Answer from the drawing. Dimensions are ordinates in mm from the lowest x, y and z of the part. A direction names the side the tool comes from. Round coordinates to 2 decimals unless told otherwise and drop trailing zeros. Loops run counter-clockwise (first coordinate to the right, second up) from the corner with the lowest first, then second, coordinate; pieces in that order, holes last.
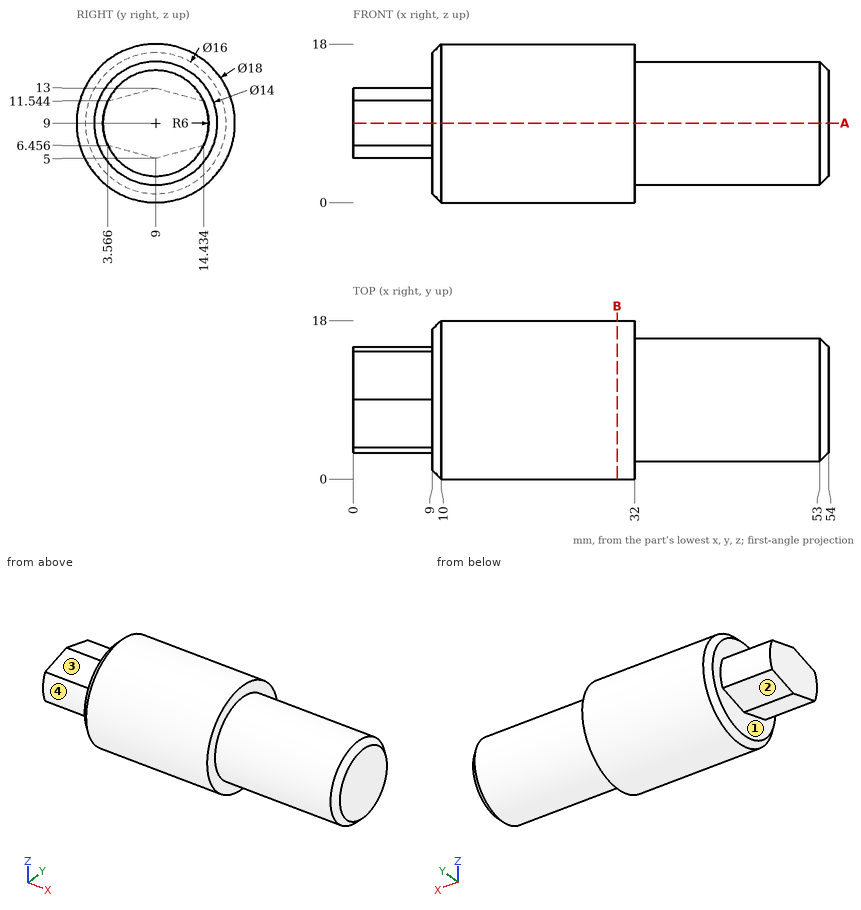
Item 1: Section A-A, the plane z = 9 is taken. Give the vertices of the cut face in (x, y).
Item 2: Straight lines are drawn through the part: line 1 (X direction, y = 3.75, z = 3); line 2 (X direction, y = 9, z = 13.25); line 3 (Y direction, x = 23.5, z = 3). For each, find the intervals that lie inside material, in ascending order.
Item 3: Section B-B, the plane x = 30 is taken. Give the vertices of the cut face in (y, z).
Item 4: For the marked faces 1, 2, 3 and 4, determine the directions among +Z, -Z, +X, -X, +Y, -Y from which every point of the face is accessible in a straight line to the end or side of a thin tool.
Item 5: Each of these flat-tipped pins is pushed along its axis until it touches: P1, Ø3, axis at y = 11, z = 12, coming from the -X side; P2, Ø5, axis at x = 19, y = 3, coming from the +Z side; P3, Ø4, axis at x = 8.5, y = 3, coming from the +Z side; P4, Ø5, axis at x = 30, z = 6, coming from the -Y side. Where does it stop, or does it pass through?
Answer below:
1. outline: (0, 3) - (9, 3) - (9, 1) - (10, 0) - (32, 0) - (32, 2) - (53, 2) - (54, 3) - (54, 15) - (53, 16) - (32, 16) - (32, 18) - (10, 18) - (9, 17) - (9, 15) - (0, 15) - close
2. line 1: x = 9 to 32
2. line 2: x = 9 to 54
2. line 3: y = 2.29 to 15.71
3. outline: circle Ø18 at (9, 9)
4. face 1: -X
4. face 2: -Z, -X, +Y
4. face 3: +Z, -X, -Y
4. face 4: -X, -Y
5. P1: stops at x = 0
5. P2: stops at z = 17.29
5. P3: stops at z = 16.69
5. P4: stops at y = 0.01
